Could you check a few things on this model? Use its own coordinates, in mm. A direction names the side the tool comes from. Coordinates: 2 decimals unless noted, no trailing zeros. Order: outer loops, then holes, each group sorted by start corner. A loop starts at its lowest first (then second) coordinate and runs counter-clockwise, first axis right, second up. Notation, with made-up numbers: (-22, 38.25) -> (-15, 38.25) arc R25 cw to (-15, 71.25) -> close; hole circle Ø7 at (22, 50). An arc over 180 degrees is marked (long way). Put each result on its own line as item: value. Start each with the question number.
Q1. Please list where these lines run through material, in increasing order: line 1 along Y through (x, z) = (10.25, 5.6); line 2 along X through (y, z) = (2.25, 3); line 3 along Y through (x, z) = (-10.25, 2.7).
Q2. If we section it at B-B (z = 1.5): Please give me the cut outline in (x, y).
Q3. Will these pins go through, and if not, where does the flat tip stop? pin 1 (2 mm diameter, centred on x = -3, y = -4, fed in from -Z); pin 2 (1.5 mm diameter, centred on x = 8.5, y = -1, fed in from -Z).
Q4. If we section it at D-D (z = 5.5): Please give me the cut outline in (x, y).
Q5. For faces 1 (the face through (12.631, -1.825, 1.676)), 2 (the face through (9.88, -1.66, 5.73)), which set-ups out of +Z, -Z, +X, -X, +Y, -Y let a thin tool reach every point of the face, with its end or its side?
Q6. We'd pull the mould along X, two halves only. Please class faces 3 (the face through (15, 0, 4)), 4 (the face through (8, 0, 3.4)), 5 (the face through (-15, 0, 4)): +X half, -X half, draft (parallel to the pull), parting line (faces both ways), or undercut.
Q7. If we section it at C-C (y = 0): Please give me the cut outline in (x, z).
Q8. If we section it at A-A (x = 10.25): Please give me the cut outline in (y, z), and give its area (3 significant figures).
from build123d import *

# Parameters (mm, degrees)
SKETCH_1_W                = 30
SKETCH_1_H                = 10
EXTRUDE_1_DEPTH           = 8
HOLE_WIZARD_1_D           = 3.4
HOLE_WIZARD_1_CBORE_D     = 6
HOLE_WIZARD_1_CBORE_DEPTH = 3.4


with BuildPart() as part:
    # 草图1 → 凸台-拉伸1 (new body)
    with BuildSketch(Plane.XY):
        Rectangle(SKETCH_1_W, SKETCH_1_H)
    extrude(amount=EXTRUDE_1_DEPTH)

    # 打孔尺寸(%根据)内六角圆柱头螺钉的类型1 (through all)
    with Locations(Plane(origin=(0, 0, 0), x_dir=(-1, 0, 0), z_dir=(0, 0, -1))):
        with Locations((-10.25, 0), (10.25, 0)):
            CounterBoreHole(HOLE_WIZARD_1_D / 2, HOLE_WIZARD_1_CBORE_D / 2, HOLE_WIZARD_1_CBORE_DEPTH)


solid = part.part
The answers:
1. line 1: -5 to -1.7, 1.7 to 5
1. line 2: -15 to -12.23, -8.27 to 8.27, 12.23 to 15
1. line 3: -5 to -3, 3 to 5
2. outline: (-15, -5) -> (15, -5) -> (15, 5) -> (-15, 5) -> close; hole circle Ø6 at (-10.25, 0); hole circle Ø6 at (10.25, 0)
3. pin 1: z = 0
3. pin 2: z = 3.4
4. outline: (-15, -5) -> (15, -5) -> (15, 5) -> (-15, 5) -> close; hole circle Ø3.4 at (-10.25, 0); hole circle Ø3.4 at (10.25, 0)
5. face 1: -Z
5. face 2: +Z, -Z
6. face 3: +X half
6. face 4: undercut
6. face 5: -X half
7. outline: (-15, 0) -> (-13.25, 0) -> (-13.25, 3.4) -> (-11.95, 3.4) -> (-11.95, 8) -> (-15, 8) -> close; (-8.55, 3.4) -> (-7.25, 3.4) -> (-7.25, 0) -> (7.25, 0) -> (7.25, 3.4) -> (8.55, 3.4) -> (8.55, 8) -> (-8.55, 8) -> close; (11.95, 3.4) -> (13.25, 3.4) -> (13.25, 0) -> (15, 0) -> (15, 8) -> (11.95, 8) -> close
8. outline: (-5, 0) -> (-3, 0) -> (-3, 3.4) -> (-1.7, 3.4) -> (-1.7, 8) -> (-5, 8) -> close; (1.7, 3.4) -> (3, 3.4) -> (3, 0) -> (5, 0) -> (5, 8) -> (1.7, 8) -> close
8. area: 44.0 mm^2
